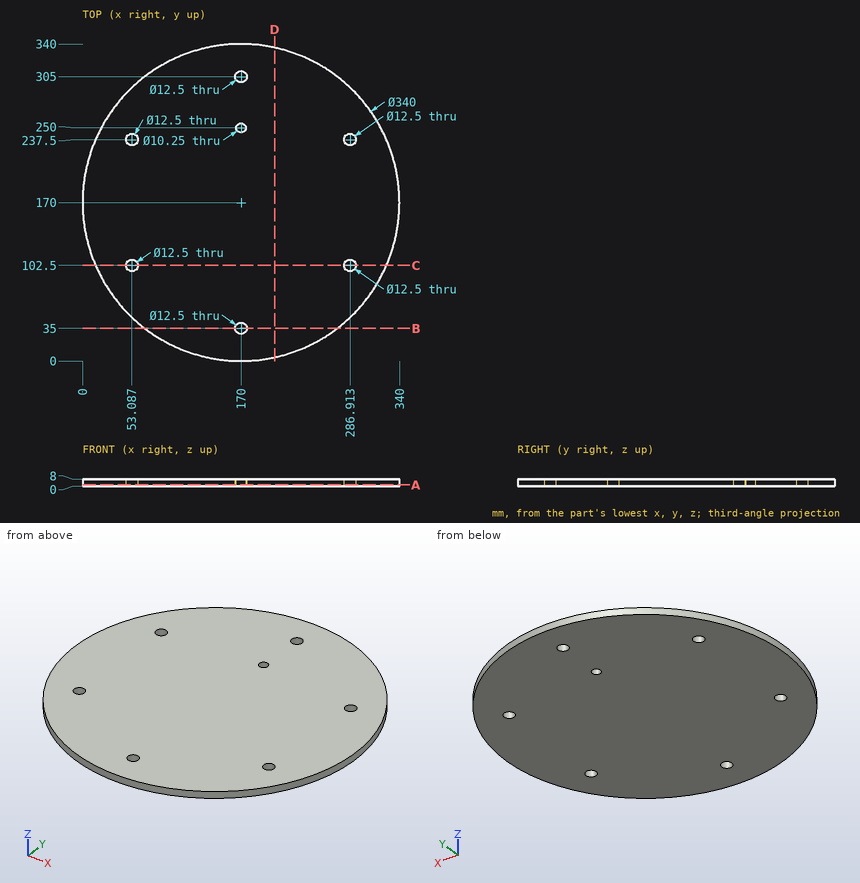
Study the drawing (mm; zero at the part's minimum x, y, z) and answer. Round coordinates to 2 decimals unless told otherwise and drop trailing zeros. Write each loop counter-clockwise with the first axis right and the second up, starting at its lowest first coordinate (ties: lowest second). Pieces come first, ordered by that corner, then holes. Notation, with made-up numbers: (-25, 0) - (15, 0) arc R30 cw to (15, 33) - close; hole circle Ø4 at (-23.75, 63). An arc over 180 degrees is marked (long way). Use a Markdown table: item, result. Add a question column.
1. A flat-ended cylindrical pin translates along its axis: P1, Ø4, axis at x = 267, z = 3, coming from the +Y side. Find the tip coordinate at first contact, or state that the pin passes through.
2. The part is cut by section C-C (y = 102.5). Write down the section's boundary in (x, z) (1 decimal).
3. Consider line 1 (Y direction, x = 288.5, z = 7.5) (1 decimal); line 2 (Y direction, x = 48, z = 2) (1 decimal); line 3 (X direction, y = 305, z = 3.25). Determine where each line is inside the solid, lowest interval first.
4. The part is cut by section A-A (z = 1.75). Give the number of separate pieces and of enclosed holes in the cut face, and give its area (3 significant figures).
5. The part is cut by section B-B (y = 35). Write down the section's boundary in (x, z).
6. The part is cut by section D-D (x = 206). Write down the section's boundary in (y, z) (1 decimal).
Reported:
| question | item | result |
|---|---|---|
| 1 | P1 | y = 310.98 |
| 2 | outline | (14, 0) - (46.8, 0) - (46.8, 8) - (14, 8) - close; (59.3, 0) - (280.7, 0) - (280.7, 8) - (59.3, 8) - close; (293.2, 0) - (326, 0) - (326, 8) - (293.2, 8) - close |
| 3 | line 1 | 48.1 to 96.5, 108.5 to 231.5, 243.5 to 291.9 |
| 3 | line 2 | 51.6 to 98.9, 106.1 to 233.9, 241.1 to 288.4 |
| 3 | line 3 | 66.68 to 163.75, 176.25 to 273.32 |
| 4 | separate pieces | 1 |
| 4 | enclosed holes | 7 |
| 4 | area | 90,000 mm^2 |
| 5 | outline | (66.68, 0) - (163.75, 0) - (163.75, 8) - (66.68, 8) - close; (176.25, 0) - (273.32, 0) - (273.32, 8) - (176.25, 8) - close |
| 6 | outline | (3.9, 0) - (336.1, 0) - (336.1, 8) - (3.9, 8) - close |
